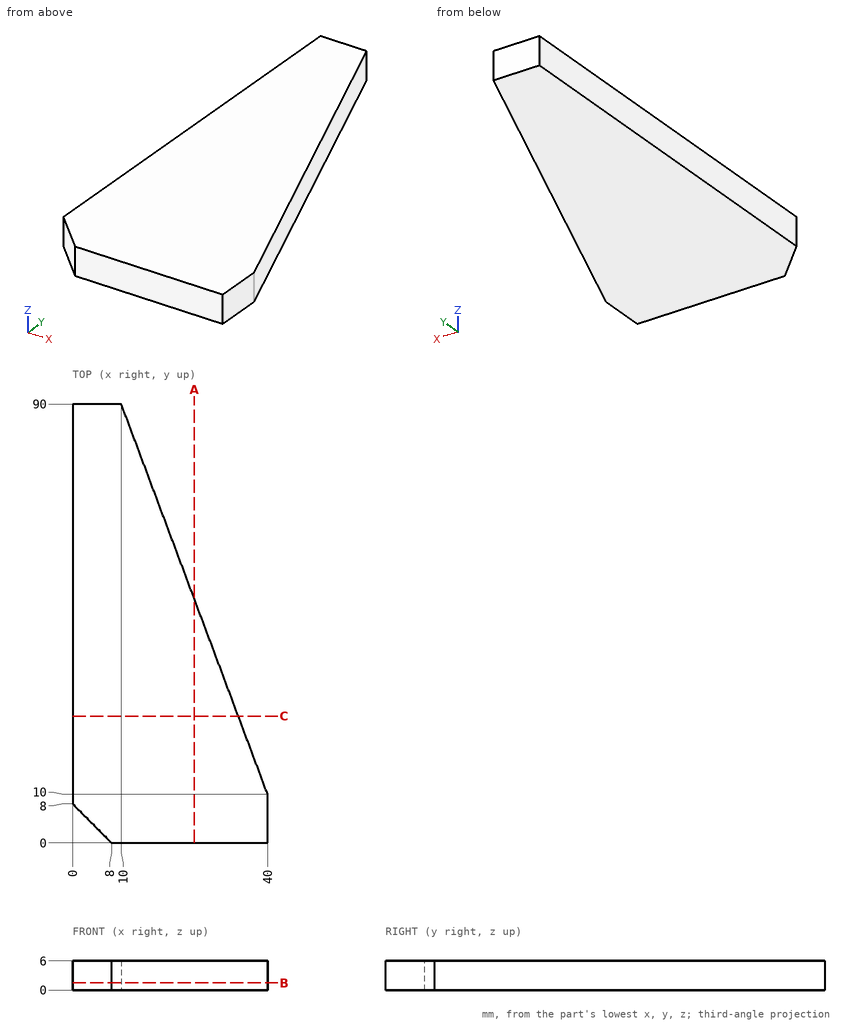
Here's the drawing with two shaded views (mm, measured from the low corner). I have some questions. Coordinates: 2 decimals unless noted, no trailing zeros. Loops run counter-clockwise (first coordinate to the right, second up) from the corner with the lowest first, then second, coordinate; pieces in that order, holes last. Notation, with made-up numbers: M 21,49 L 65,49 A19 cw 65,55 Z; hole C 22.25,63.25 d1. An arc over 180 degrees is marked long. Answer as CSV lines item,"result". Start each with the question number.
1. Suppose I cut it at A-A, the plane x = 25. List the corners of the cut face in (y, z) for me, plus the area to 3 significant figures.
2. Suppose I cut it at B-B, the plane z = 1.5. List the corners of the cut face in (x, y) for me.
3. If I drill on probe 1 along X at (y, z) = (27, 2) (3 decimals); probe 2 along X at (y, z) = (42, 0.75); probe 3 along Y at (x, z) = (5.5, 3.75), over which ranges is the centre line in solid material (lowest first)? Write a range as [from, to].
4. Suppose I cut it at C-C, the plane y = 26. List the corners of the cut face in (x, z) for me, plus the area to 3 significant figures.
Output:
1,outline,"M 0,0 L 50,0 L 50,6 L 0,6 Z"
1,area,"300 mm^2"
2,outline,"M 0,8 L 8,0 L 40,0 L 40,10 L 10,90 L 0,90 Z"
3,probe 1,"x = [0, 33.625]"
3,probe 2,"x = [0, 28]"
3,probe 3,"y = [2.5, 90]"
4,outline,"M 0,0 L 34,0 L 34,6 L 0,6 Z"
4,area,"204 mm^2"
